For this review, take the finished solid that the model builds, in its own axes (mm). A direction names the side the tool comes from. Give positions to 0.01 mm unless a question says otherwise; leave off trailing zeros. Order: outer loops, then holes, each group sorted by start corner. A loop starts at its lowest first (then second) coordinate and runs counter-clockwise, first axis right, second up. Notation, with made-up numbers: (-28, 40.25) -> (22, 40.25) arc R21 cw to (22, 51.25) -> close; hole circle Ø8 at (-23, -33). An arc over 180 degrees is marked (long way). One line per item, written item: value. Start each with the question number.
from build123d import *
from build123d.topology import SkipClean

# Parameters (mm, degrees)
MAIN_BODY_PLATE_DEPTH   = 12
UPPER_HUB_SKETCH_R      = 15
UPPER_HUB_30_DEPTH      = 6
SPACER_BLOCK_SKETCH_W   = 38
SPACER_BLOCK_SKETCH_H   = 50
SPACER_BLOCK_DEPTH      = 12
LOWER_LUG_DEPTH         = 12
LOWER_START             = 6
LOWER_HUB_SKETCH_R      = 15
LOWER_HUB_30_DEPTH      = 6
LOWER_PIN_BORE_SKETCH_R = 7
LOWER_PIN_BORE_14_DEPTH = 18
UPPER_START             = -18
UPPER_PIN_BORE_SKETCH_R = 7
UPPER_PIN_BORE_14_DEPTH = 18
CLEVIS_PLATE_DEPTH      = 12
CLEVIS_HUB_SKETCH_R     = 12.5
CLEVIS_HUB_25_DEPTH     = 10
CLEVIS_START            = -12
CLEVIS_WEB_DEPTH        = 12
CLEVIS_START_2          = -20
CLEVIS_LUG_SKETCH_R     = 12.5
CLEVIS_LUG_25_DEPTH     = 20
CLEVIS_BORE_A_SKETCH_R  = 9
CLEVIS_BORE_A_18_DEPTH  = 22
CLEVIS_START_3          = -22
CLEVIS_BORE_B_SKETCH_R  = 9
CLEVIS_BORE_B_18_DEPTH  = 22


with BuildPart() as part:
    # Main Body Profile Sketch → Main Body Plate (new body)
    with BuildSketch(Plane.XY):
        with BuildLine():
            Line((0, 0), (0, 50))
            Line((0, 50), (12, 50))
            Line((12, 50), (12, 44))
            Line((12, 44), (37, 44))
            Line((37, 44), (37, 50))
            Line((37, 50), (50, 50))
            ThreePointArc((50, 50), (75, 25), (50, 0))
            Line((50, 0), (37, 0))
            Line((37, 0), (37, 6))
            Line((37, 6), (12, 6))
            Line((12, 6), (12, 0))
            Line((12, 0), (0, 0))
        make_face()
    extrude(amount=MAIN_BODY_PLATE_DEPTH)

    # Upper Hub Sketch → Upper Hub Ø30 (add)
    with BuildSketch(Plane.XY.offset(12)):
        with Locations((50, 25)):
            Circle(UPPER_HUB_SKETCH_R)
    extrude(amount=UPPER_HUB_30_DEPTH)

    # Spacer Block Sketch → Spacer Block (add)
    with BuildSketch(Plane.ZY):
        with Locations((-19, 25)):
            Rectangle(SPACER_BLOCK_SKETCH_W, SPACER_BLOCK_SKETCH_H)
    extrude(amount=-SPACER_BLOCK_DEPTH)

    # Lower Lug Sketch → Lower Lug (add)
    with BuildSketch(Plane(origin=(0, 0, -38), x_dir=(-1, 0, 0), z_dir=(0, 0, -1))):
        with BuildLine():
            Line((-12, 44), (-37, 44))
            Line((-37, 44), (-37, 50))
            Line((-37, 50), (-50, 50))
            ThreePointArc((-50, 50), (-75, 25), (-50, 0))
            Line((-50, 0), (-37, 0))
            Line((-37, 0), (-37, 6))
            Line((-37, 6), (-12, 6))
            Line((-12, 6), (-12, 44))
        make_face()
    extrude(amount=-LOWER_LUG_DEPTH)

    # Lower Hub Sketch → Lower Hub Ø30 (add)
    with BuildSketch(Plane(origin=(0, 0, -38), x_dir=(-1, 0, 0), z_dir=(0, 0, -1)).offset(LOWER_START)):
        with Locations(Location((-50, 25, 0), (0, 0, 180))):
            Circle(LOWER_HUB_SKETCH_R)
    extrude(amount=-LOWER_HUB_30_DEPTH)

    # Lower Pin Bore Sketch → Lower Pin Bore Ø14 (cut)
    with BuildSketch(Plane(origin=(0, 0, -44), x_dir=(-1, 0, 0), z_dir=(0, 0, -1))):
        with Locations((-50, 25)):
            Circle(LOWER_PIN_BORE_SKETCH_R)
    extrude(amount=-LOWER_PIN_BORE_14_DEPTH, mode=Mode.SUBTRACT)

    # Upper Pin Bore Sketch → Upper Pin Bore Ø14 (cut)
    with BuildSketch(Plane.XY.offset(18).offset(UPPER_START)):
        with Locations(Location((50, 25, 0), (0, 0, 180))):
            Circle(UPPER_PIN_BORE_SKETCH_R)
    extrude(amount=UPPER_PIN_BORE_14_DEPTH, mode=Mode.SUBTRACT)

    # Clevis Plate Sketch → Clevis Plate (add)
    with BuildSketch(Plane(origin=(0, 50, 0), x_dir=(1, 0, 0), z_dir=(0, 1, 0))):
        with BuildLine():
            Line((0, 38), (-30.142972847, 24.392972847))
            ThreePointArc((-30.142972847, 24.392972847), (-37.5, 13), (-30.142972847, 1.607027153))
            Line((-30.142972847, 1.607027153), (0, -12))
            Line((0, -12), (0, 38))
        make_face()
    extrude(amount=-CLEVIS_PLATE_DEPTH)

    # Clevis Hub Sketch → Clevis Hub Ø25 (add)
    with SkipClean():  # the faces are left unmerged after this step: merging them gives an invalid solid
        with BuildSketch(Plane.XZ.offset(-38)):
            with Locations(Location((-25, -13, 0), (0, 0, 114.295188945))):
                Circle(CLEVIS_HUB_SKETCH_R)
        extrude(amount=CLEVIS_HUB_25_DEPTH)

    # Clevis Web Sketch → Clevis Web (add)
    with SkipClean():  # the faces are left unmerged after this step: merging them gives an invalid solid
        with BuildSketch(Plane.XZ.offset(CLEVIS_START)):
            with BuildLine():
                Line((0, -38), (0, 12))
                Line((0, 12), (-30.142972847, -1.607027153))
                ThreePointArc((-30.142972847, -1.607027153), (-18.219039913, -2.499115261), (-12.5, -13))
                ThreePointArc((-12.5, -13), (-18.219039913, -23.500884739), (-30.142972847, -24.392972847))
                Line((-30.142972847, -24.392972847), (0, -38))
            make_face()
        extrude(amount=CLEVIS_WEB_DEPTH)

    # Clevis Lug Sketch → Clevis Lug Ø25 (add)
    with SkipClean():  # the faces are left unmerged after this step: merging them gives an invalid solid
        with BuildSketch(Plane.XZ.offset(CLEVIS_START_2)):
            with Locations(Location((-25, -13, 0), (0, 0, 114.295188945))):
                Circle(CLEVIS_LUG_SKETCH_R)
        extrude(amount=CLEVIS_LUG_25_DEPTH)

    # Clevis Bore A Sketch → Clevis Bore A Ø18 (cut)
    with SkipClean():  # the faces are left unmerged after this step: merging them gives an invalid solid
        with BuildSketch(Plane(origin=(0, 50, 0), x_dir=(1, 0, 0), z_dir=(0, 1, 0))):
            with Locations(Location((-25, 13, 0), (0, 0, 270))):
                Circle(CLEVIS_BORE_A_SKETCH_R)
        extrude(amount=-CLEVIS_BORE_A_18_DEPTH, mode=Mode.SUBTRACT)

    # Clevis Bore B Sketch → Clevis Bore B Ø18 (cut)
    with SkipClean():  # the faces are left unmerged after this step: merging them gives an invalid solid
        with BuildSketch(Plane.XZ.offset(CLEVIS_START_3)):
            with Locations(Location((-25, -13, 0), (0, 0, 90))):
                Circle(CLEVIS_BORE_B_SKETCH_R)
        extrude(amount=CLEVIS_BORE_B_18_DEPTH, mode=Mode.SUBTRACT)


solid = part.part
Q1. Take a section at D-D (z = -13). State the section outline as (x, y) points, and give its area (3 significant figures).
Q2. Take a section at A-A (y = 36.5). State the section outline as (x, z) points, and give its area (3 significant figures).
Q3. For faces 1 (the flat face through (30, 25, 12)), 2 (the flat face through (37, 3, -32)), 3 (the flat face through (37, 47, -32)), list the 3-axis set-ups (+Z, -Z, +X, -X, +Y, -Y) from which the entire face can be reached by the end or side of a thin tool; tool diameter is ignored.
Q4. For line 1 along X through (y, z) = (10, -13); line 2 along X through (y, z) = (25, 8.5); line 3 along Z through (x, y) = (23, 32.5), list the stretches that pass through material, from the lowest coordinate up.
Q5. For pin 1 Ø4 at (x, y) = (26.5, 5) entering from +Z; pin 2 Ø3 at (x, z) = (15.5, -37) entering from -Y; pin 3 Ø6.5 at (y, z) = (2, 4) entering from -X, all flat-tipped, find the tip position at first contact; note any pin that passes through.
Q6. Take a section at B-B (y = 25). State the section outline as (x, z) points.
Q7. Take a section at C-C (x = -17.5). State the section outline as (y, z) points.
Q8. Mouldability with a two-part tool opening along X and no side actions: class faces 4 (the flat face through (37, 47, 6)), 5 (the flat face through (43, 50, -32)), 6 (the cylindrical face through (74.994, 25.55, 5.916)) as pulls with the +X half, pulls with the -X half, needs draft (parallel to the pull), parting line crosses it, or undercut.
Answers below:
1. outline: (-37.5, 0) -> (-34, 0) -> (-34, 20) -> (-37.5, 20) -> close; (-37.5, 28) -> (-34, 28) -> (-34, 50) -> (-37.5, 50) -> close; (-16, 0) -> (12, 0) -> (12, 50) -> (-16, 50) -> (-16, 28) -> (-12.5, 28) -> (-12.5, 38) -> (0, 38) -> (0, 12) -> (-12.5, 12) -> (-12.5, 20) -> (-16, 20) -> close
1. area: 1,190 mm²
2. outline: circle Ø25 at (-25, -13); (0, -38) -> (40.37, -38) -> (40.37, -44) -> (59.63, -44) -> (59.63, -38) -> (72.2, -38) -> (72.2, -26) -> (12, -26) -> (12, 0) -> (72.2, 0) -> (72.2, 12) -> (59.63, 12) -> (59.63, 18) -> (40.37, 18) -> (40.37, 12) -> (0, 12) -> close; hole circle Ø18 at (-25, -13)
2. area: 2,510 mm²
3. face 1: +Z
3. face 2: +Z, -Z, -Y
3. face 3: +Z, -Z, +Y
4. line 1: x = -37.5 to -34, -16 to 12
4. line 2: x = 0 to 43, 57 to 75
4. line 3: z = -38 to -26, 0 to 12
5. pin 1: stops at z = 12
5. pin 2: stops at y = 6
5. pin 3: stops at x = -24.92
6. outline: (0, -38) -> (35, -38) -> (35, -44) -> (43, -44) -> (43, -26) -> (12, -26) -> (12, 0) -> (43, 0) -> (43, 18) -> (35, 18) -> (35, 12) -> (0, 12) -> close; (57, -44) -> (65, -44) -> (65, -38) -> (75, -38) -> (75, -26) -> (57, -26) -> close; (57, 0) -> (75, 0) -> (75, 12) -> (65, 12) -> (65, 18) -> (57, 18) -> close
7. outline: (0, -30.1) -> (12, -30.1) -> (12, -23) -> (20, -23) -> (20, -17.97) -> (0, -17.97) -> close; (0, -8.03) -> (20, -8.03) -> (20, -3) -> (12, -3) -> (12, 4.1) -> (0, 4.1) -> close; (28, -23) -> (38, -23) -> (38, -30.1) -> (50, -30.1) -> (50, -17.97) -> (28, -17.97) -> close; (28, -8.03) -> (50, -8.03) -> (50, 4.1) -> (38, 4.1) -> (38, -3) -> (28, -3) -> close
8. face 4: undercut
8. face 5: needs draft
8. face 6: pulls with the +X half
